The model under review builds one solid part; all positions refer to its coordinate system, in mm. Give positions to 0.01 mm unless a question says otherwise; leave off trailing zeros. Loops run counter-clockwise (first coordinate to the right, second up) from the corner with the lowest first, then second, coordinate; pieces in that order, holes last. Notation, with made-up numbers: (51.25, 13.5) - (93.25, 13.5) arc R13 cw to (93.25, 26.5) - close; hole circle Ø5 at (21.5, -19.5). An arc over 180 degrees is marked (long way). Answer as a JSON object with one key per item and string values.
from build123d import *

# Parameters (mm, degrees)
SKETCH12_W                = 20
SKETCH12_H                = 20
SKETCH12_W_2              = 18
SKETCH12_H_2              = 18
F_20_X_20_X_1_1_DEPTH     = 1300
HOLE_WIZARD_10_5_10_5_1_D = 10.5


with BuildPart() as part:
    # Sketch12 → 方通 20 X 20 X 1(1) (new body)
    with BuildSketch(Plane.ZX):
        Rectangle(SKETCH12_W, SKETCH12_H)
        Rectangle(SKETCH12_W_2, SKETCH12_H_2, mode=Mode.SUBTRACT)
    extrude(amount=F_20_X_20_X_1_1_DEPTH)

    # Ø10.5 (10.5) 直径孔1 (through all)
    with Locations(Plane(origin=(10, 0, 0), x_dir=(0, 0, -1), z_dir=(1, 0, 0))):
        with Locations((0, 20), (0, 1280)):
            Hole(HOLE_WIZARD_10_5_10_5_1_D / 2)


solid = part.part
Q1. Consider section A-A, the plane y = 1054.5. State the section outline as (x, z) points.
Results:
{"outline": "(-10, -10) - (10, -10) - (10, 10) - (-10, 10) - close; hole (-9, -9) - (9, -9) - (9, 9) - (-9, 9) - close"}
Q2. To check wall thickness, follow probe 1 along Y at (x, z) = (-9.45, 0); probe 2 along Z at (x, y) = (5, 304.5). State the ranges of each line that lie inside material, in increasing order. Write a range as [from, to].
Results:
{"probe 1": "y = [0, 14.75], [25.25, 1274.75], [1285.25, 1300]", "probe 2": "z = [-10, -9], [9, 10]"}
Q3. Clearance check with a flat-ended pin moving along its axis: pin 1 Ø6.5 at (y, z) = (1280, 0) entering from -X (3 decimals). State where the tip first meets the part, or that it passes through.
Results:
{"pin 1": "passes through"}
Q4. Consider section B-B, the plane z = 0. State the section outline as (x, y) points, plus the area to 3 significant figures.
Results:
{"outline": "(-10, 0) - (-9, 0) - (-9, 14.75) - (-10, 14.75) - close; (-10, 25.25) - (-9, 25.25) - (-9, 1274.75) - (-10, 1274.75) - close; (-10, 1285.25) - (-9, 1285.25) - (-9, 1300) - (-10, 1300) - close; (9, 0) - (10, 0) - (10, 14.75) - (9, 14.75) - close; (9, 25.25) - (10, 25.25) - (10, 1274.75) - (9, 1274.75) - close; (9, 1285.25) - (10, 1285.25) - (10, 1300) - (9, 1300) - close", "area": "2,560 mm^2"}
